Can you work these out from the model? Positions are in its coordinate system, mm. Give positions to 0.01 mm unless a question says otherwise; leave off trailing zeros. Order: outer loops, then holes, each group sorted by start corner. A loop starts at its lowest first (then second) coordinate and runs counter-clockwise, first axis right, second up.
```python
from build123d import *

# Parameters (mm, degrees)
SKETCH1_W           = 144
SKETCH1_H           = 70
SKETCH1_R           = 3.5
BOSS_EXTRUDE1_DEPTH = 8
CHAMFER1_SIZE       = 2
M6_TAPPED_HOLE1_D   = 5


with BuildPart() as part:
    # Sketch1 → Boss-Extrude1 (new body)
    with BuildSketch(Plane.XY):
        Rectangle(SKETCH1_W, SKETCH1_H)
        with Locations((65, 30)):
            Circle(SKETCH1_R, mode=Mode.SUBTRACT)
        with Locations((65, -30)):
            Circle(SKETCH1_R, mode=Mode.SUBTRACT)
        with Locations((-65, -30)):
            Circle(SKETCH1_R, mode=Mode.SUBTRACT)
        with Locations((-65, 30)):
            Circle(SKETCH1_R, mode=Mode.SUBTRACT)
    extrude(amount=BOSS_EXTRUDE1_DEPTH)

    # Chamfer1
    chamfer1_edges = [part.edges().sort_by_distance(p)[0] for p in [
        (-72, -35, 4),
        (-72, 35, 4),
        (72, 35, 4),
        (72, -35, 4),
    ]]
    chamfer(chamfer1_edges, length=CHAMFER1_SIZE)

    # M6 Tapped Hole1 (through all)
    with Locations(Plane.XY.offset(8)):
        with Locations((-52.5, 30), (-52.5, -30), (52.5, -30), (52.5, 30)):
            Hole(M6_TAPPED_HOLE1_D / 2)


solid = part.part
```
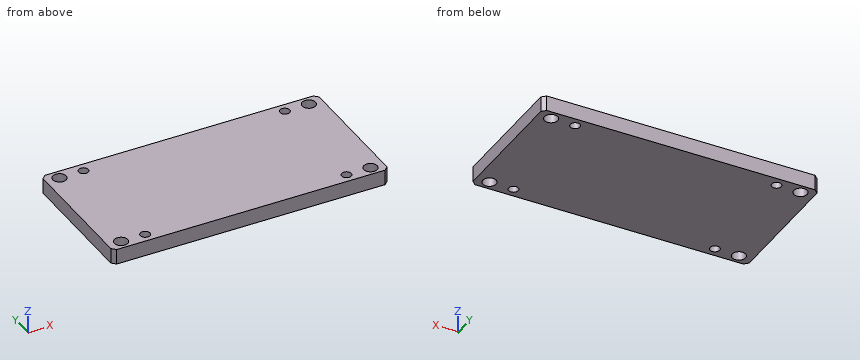
1) I'm going to push a flat-ended pin straight in: pin 1 Ø9 at (x, y) = (65, -30) entering from +Z. Where does the tip first touch, or does it pass through?
2) If I drill on line 1 (Y direction, x = -65, z = 5.25); line 2 (Y direction, x = -52.5, z = 2.5), over which ranges is the centre line in solid material (lowest first)?
3) Suppose I cut it at B-B (x = 52). Please give me the cut outline in (y, z).
4) Suppose I cut it at C-C (z = 5). Give the number of separate pieces and of enclosed holes in the cut face, and give its area (3 significant figures).
5) Suppose I cut it at A-A (y = -30). Please give me the cut outline in (x, z).
Results:
1. pin 1: stops at z = 8
2. line 1: y = -35 to -33.5, -26.5 to 26.5, 33.5 to 35
2. line 2: y = -35 to -32.5, -27.5 to 27.5, 32.5 to 35
3. outline: (-35, 0) - (-32.45, 0) - (-32.45, 8) - (-35, 8) - close; (-27.55, 0) - (27.55, 0) - (27.55, 8) - (-27.55, 8) - close; (32.45, 0) - (35, 0) - (35, 8) - (32.45, 8) - close
4. separate pieces: 1
4. enclosed holes: 8
4. area: 9,840 mm2
5. outline: (-72, 0) - (-68.5, 0) - (-68.5, 8) - (-72, 8) - close; (-61.5, 0) - (-55, 0) - (-55, 8) - (-61.5, 8) - close; (-50, 0) - (50, 0) - (50, 8) - (-50, 8) - close; (55, 0) - (61.5, 0) - (61.5, 8) - (55, 8) - close; (68.5, 0) - (72, 0) - (72, 8) - (68.5, 8) - close
